from build123d import *

# Parameters (mm, degrees)
EXTRUDE_1_DEPTH = 1650
SKETCH_2_R      = 4
EXTRUDE_2_DEPTH = 30


with BuildPart() as part:
    # 草图1 → 凸台-拉伸1 (new body)
    with BuildSketch(Plane(origin=(0, 0, 0), x_dir=(1, 0, 0), z_dir=(0, 1, 0))):
        with BuildLine():
            Line((-16, -10), (16, -10))
            ThreePointArc((16, -10), (18.828427125, -8.828427125), (20, -6))
            Line((20, -6), (20, 6))
            ThreePointArc((20, 6), (18.828427125, 8.828427125), (16, 10))
            Line((16, 10), (-16, 10))
            ThreePointArc((-16, 10), (-18.828427125, 8.828427125), (-20, 6))
            Line((-20, 6), (-20, -6))
            ThreePointArc((-20, -6), (-18.828427125, -8.828427125), (-16, -10))
        make_face()
        with BuildLine():
            Line((-16, -8), (16, -8))
            ThreePointArc((16, -8), (17.414213562, -7.414213562), (18, -6))
            Line((18, -6), (18, 6))
            ThreePointArc((18, 6), (17.414213562, 7.414213562), (16, 8))
            Line((16, 8), (-16, 8))
            ThreePointArc((-16, 8), (-17.414213562, 7.414213562), (-18, 6))
            Line((-18, 6), (-18, -6))
            ThreePointArc((-18, -6), (-17.414213562, -7.414213562), (-16, -8))
        make_face(mode=Mode.SUBTRACT)
    extrude(amount=EXTRUDE_1_DEPTH)

    # 草图2 → 凸台-拉伸2 (add)
    with BuildSketch(Plane(origin=(0, 0, -10), x_dir=(-1, 0, 0), z_dir=(0, 0, -1))):
        with Locations(Location((0, 1625, 0), (0, 0, 180))):
            Circle(SKETCH_2_R)
        with Locations(Location((0, 25, 0), (0, 0, 180))):
            Circle(SKETCH_2_R)
    extrude(amount=EXTRUDE_2_DEPTH)


solid = part.part
Could you check a few things on this model? Use its own coordinates, in mm. Give positions to 0.01 mm unless a question says otherwise; leave off trailing zeros. Write each loop counter-clockwise with the first axis right and the second up, starting at its lowest first coordinate (ties: lowest second). Pieces come first, ordered by that corner, then holes. Notation, with made-up numbers: (24, 73.5) -> (81, 73.5) arc R22 ccw to (81, 100.5) -> close; hole circle Ø11 at (81.25, -30.75). An arc over 180 degrees is marked (long way). Answer as CSV lines item,"result". Start each with the question number.
(1) Please list where these lines run through material, in increasing order: line 1 (X direction, y = 583.5, z = 6); line 2 (Z direction, x = 2.5, y = 81); line 3 (X direction, y = 1316, z = 7).
(2) I'm going to push flat-ended pins straight in: pin 1 Ø10 at (x, z) = (-9.5, -1) entering from -Y; pin 2 Ø8 at (x, z) = (-14.5, -4.5) entering from -Y; pin 3 Ø12 at (x, z) = (9, -24.5) entering from -Y; pin 4 Ø3 at (x, y) = (-2, 1283) entering from -Z. Where does each tip first touch, or does it pass through?
(3) If we mould it in two halves opening along Z, with no side actions, what happens to faces 1 (the face through (0, 813, 10)), 2 (the face through (0, 813, -8)), 3 (the face through (0, 813, -10))? For each: +Z half, -Z half, draft (parallel to the pull), parting line (faces both ways), or undercut.
(4) If we section it at B-B, the plane y = 819: Write out the boundary of the cut face in (x, z).
(5) If we section it at A-A, the plane z = -28.5: Write out the boundary of the cut face in (x, y), and give its area (3 significant figures).
Answer list:
1,line 1,"-20 to -18, 18 to 20"
1,line 2,"-10 to -8, 8 to 10"
1,line 3,"-19.87 to -17.73, 17.73 to 19.87"
2,pin 1,"through"
2,pin 2,"y = 0"
2,pin 3,"y = 22.35"
2,pin 4,"z = -10"
3,face 1,"+Z half"
3,face 2,"undercut"
3,face 3,"-Z half"
4,outline,"(-20, -6) arc R4 ccw to (-16, -10) -> (16, -10) arc R4 ccw to (20, -6) -> (20, 6) arc R4 ccw to (16, 10) -> (-16, 10) arc R4 ccw to (-20, 6) -> close; hole (-18, -6) arc R2 ccw to (-16, -8) -> (16, -8) arc R2 ccw to (18, -6) -> (18, 6) arc R2 ccw to (16, 8) -> (-16, 8) arc R2 ccw to (-18, 6) -> close"
5,outline,"circle Ø8 at (0, 25); circle Ø8 at (0, 1625)"
5,area,"101 mm^2"
